Input: part model. Units: mm. Frame: model coordinates. A direction names the side the tool comes from. Round coordinates to 2 decimals unless told otherwise and drop trailing zeros. Write each loop counter-clockwise with the first axis right and the second up, starting at its lowest first coordinate (ties: lowest second). Pieces come first, ordered by that corner, then holes. Notation, with made-up numbers: M -7.5,56.25 L 16.5,56.25 A14 ccw 16.5,62.25 Z; hole C 41.5,-20.75 d4. An arc over 180 degrees is marked long. Answer as CSV lines item,"result". Start each with the question number.
```python
from build123d import *

# Parameters (mm, degrees)
BOSS_EXTRUDE1_DEPTH = 7.5
SKETCH3_R           = 6
BOSS_EXTRUDE2_DEPTH = 140
CHAMFER1_SIZE       = 1.2


with BuildPart() as part:
    # Sketch1 → Boss-Extrude1 (new body)
    with BuildSketch(Plane.XY):
        Polygon((9, 5.196152423), (0, 10.392304845), (-9, 5.196152423), (-9, -5.196152423), (0, -10.392304845), (9, -5.196152423), align=None)
    extrude(amount=BOSS_EXTRUDE1_DEPTH)

    # Sketch3 → Boss-Extrude2 (add)
    with BuildSketch(Plane.XY.offset(7.5)):
        Circle(SKETCH3_R)
    extrude(amount=BOSS_EXTRUDE2_DEPTH)

    # Chamfer1
    chamfer1_edges = [part.edges().sort_by_distance(p)[0] for p in [
        (-6, 0, 147.5),
    ]]
    chamfer(chamfer1_edges, length=CHAMFER1_SIZE)


solid = part.part
```
Item 1: Line query: line 1 (Z direction, x = -3.75, y = 6.5); line 2 (Y direction, x = 0, z = 119); line 3 (Y direction, x = -4.5, z = 96). Output: solid intervals per line, ascending. Write a range as [from, to].
Item 2: Cut plane A-A, the plane y = 0. Return loops of the section in (x, z), plus the area to 3 significant figures.
Item 3: Cut plane B-B, the plane z = 68.5. Return loops of the section in (x, y).
Item 4: Cut plane C-C, the plane y = 8.5. Return loops of the section in (x, z), plus the area to 3 significant figures.
Item 5: Pin query (flat end, axial travel): pin 1 Ø3 at (x, z) = (1, 70) entering from -Y; pin 2 Ø2 at (y, z) = (4, 35) entering from -X; pin 3 Ø5 at (x, z) = (-6, 88) entering from +Y. Return the tip coordinate at first contact, or that it passes through.
Item 6: Access query for faces 1 (the face through (-6, 0, 76)), 2 (the face through (0, 0, 147.5)). Directions: +Z, -Z, +X, -X, +Y, -Y. A direction counts if a zero-diameter tool reaches every point of the face in a straight line with its end or side. Return the directions, or none.
Item 7: Cut plane D-D, the plane y = -7.25. Return loops of the section in (x, z), plus the area to 3 significant figures.
Results list:
1,line 1,"[0, 7.5]"
1,line 2,"[-6, 6]"
1,line 3,"[-3.97, 3.97]"
2,outline,"M -9,0 L 9,0 L 9,7.5 L 6,7.5 L 6,146.3 L 4.8,147.5 L -4.8,147.5 L -6,146.3 L -6,7.5 L -9,7.5 Z"
2,area,"1,810 mm²"
3,outline,"C 0,0 d12"
4,outline,"M -3.28,0 L 3.28,0 L 3.28,7.5 L -3.28,7.5 Z"
4,area,"49.2 mm²"
5,pin 1,"y = -6"
5,pin 2,"x = -5.2"
5,pin 3,"y = 4.87"
6,face 1,"+Z"
6,face 2,"+Z, +X, -X, +Y, -Y"
7,outline,"M -5.44,0 L 5.44,0 L 5.44,7.5 L -5.44,7.5 Z"
7,area,"81.6 mm²"
